Can you work these out from the drawing? Everything is in mm from the part's minimum corner. A direction names the side the tool comes from. Give positions to 0.01 mm unless a question says otherwise; leave off trailing zeros. Write each loop counter-clockwise with the first axis right and the second up, starting at its lowest first coordinate (ties: lowest second). Pieces come first, ordered by that corner, then holes. Notation, with made-up numbers: (-19, 47) - (39, 47) arc R23 ccw to (39, 72) - close; hole circle Ø4 at (21.25, 80.25). An arc over 180 degrees is marked (long way). Write each question's results on one line, items separated by ' | '. Start each with the question number.
Item 1: Suppose I cut it at D-D on x = 31. List the corners of the cut face in (y, z) for me.
Item 2: Suppose I cut it at A-A on x = 15. List the corners of the cut face in (y, z) for me, then the cut area to 3 significant figures.
Item 3: Suppose I cut it at B-B on z = 5. List the corners of the cut face in (x, y) for me, then the cut area to 3 significant figures.
Item 4: Will these pins go through, and if not, where does the flat tip stop? P1, Ø1.9, axis at x = 30, z = 5, coming from the -Y side; P2, Ø5, axis at x = 15, z = 5, coming from the +Y side.
Item 5: Suppose I cut it at C-C on y = 1. List the corners of the cut face in (x, z) for me, then the cut area to 3 significant figures.
Item 6: We'd pull the mould along X, two halves only. Please class the marked faces 3, 4 and 5: +X half, -X half, draft (parallel to the pull), parting line (faces both ways), or undercut.
Item 7: Please list where these lines run through material, in increasing order: line 1 along X through (y, z) = (2.25, 5); line 2 along Z through (x, y) = (30, 6.7); line 3 along Z through (x, y) = (30, 1.2).
Item 8: Which directions (+Z, -Z, +X, -X, +Y, -Y) give clear straight access to the entire face, cutting with the end or side of a thin tool? Please do the marked faces 1 and 2.
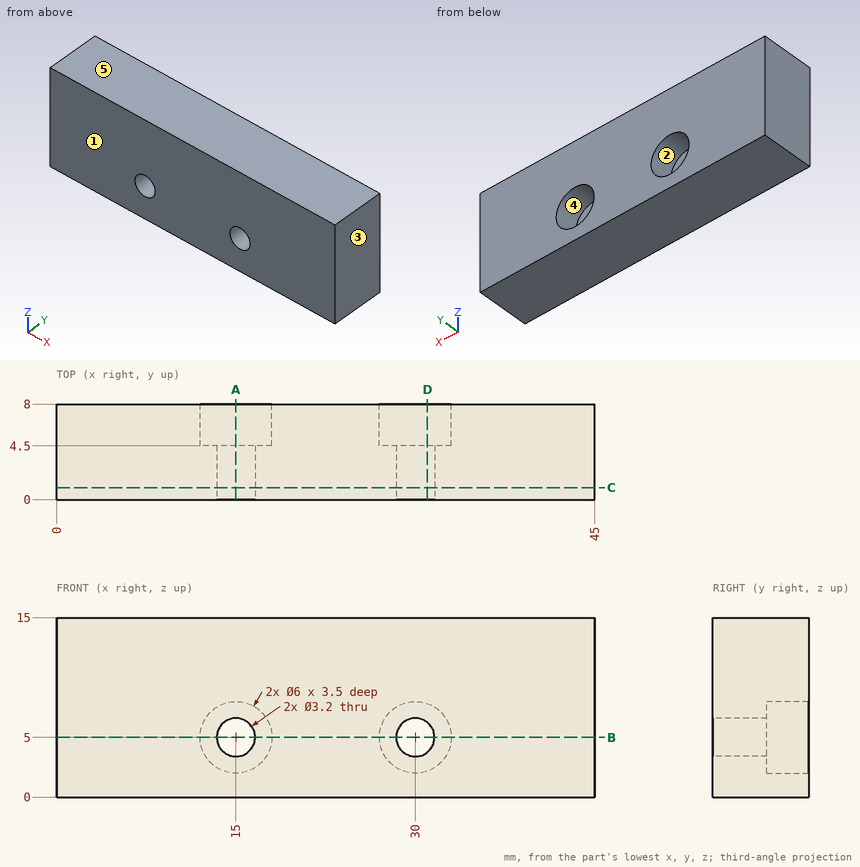
Checked values:
1) outline: (0, 0) - (8, 0) - (8, 2.17) - (4.5, 2.17) - (4.5, 3.75) - (0, 3.75) - close; (0, 6.25) - (4.5, 6.25) - (4.5, 7.83) - (8, 7.83) - (8, 15) - (0, 15) - close
2) outline: (0, 0) - (8, 0) - (8, 2) - (4.5, 2) - (4.5, 3.4) - (0, 3.4) - close; (0, 6.6) - (4.5, 6.6) - (4.5, 8) - (8, 8) - (8, 15) - (0, 15) - close | area: 84.6 mm^2
3) outline: (0, 0) - (13.4, 0) - (13.4, 4.5) - (12, 4.5) - (12, 8) - (0, 8) - close; (16.6, 0) - (28.4, 0) - (28.4, 4.5) - (27, 4.5) - (27, 8) - (18, 8) - (18, 4.5) - (16.6, 4.5) - close; (31.6, 0) - (45, 0) - (45, 8) - (33, 8) - (33, 4.5) - (31.6, 4.5) - close | area: 289 mm^2
4) P1: passes through | P2: stops at y = 4.5
5) outline: (0, 0) - (45, 0) - (45, 15) - (0, 15) - close; hole circle Ø3.2 at (15, 5); hole circle Ø3.2 at (30, 5) | area: 659 mm^2
6) face 3: +X half | face 4: undercut | face 5: draft
7) line 1: x = 0 to 13.4, 16.6 to 28.4, 31.6 to 45 | line 2: z = 0 to 2, 8 to 15 | line 3: z = 0 to 3.4, 6.6 to 15
8) face 1: +Z, -Z, +X, -X, -Y | face 2: +Y
